from build123d import *

# Parameters (mm, degrees)
BOSS_EXTRUDE1_DEPTH = 6
SKETCH2_W           = 2.25
SKETCH2_H           = 2
CUT_EXTRUDE1_DEPTH  = 9.628586211
SKETCH3_W           = 2.25
SKETCH3_H           = 2
CUT_EXTRUDE2_DEPTH  = 9.628586211
SKETCH4_W           = 2.5
SKETCH4_H           = 50
CHAMFER1_SIZE       = 0.4905
FILLET1_R           = 0.5
FILLET2_R           = 3


with BuildPart() as part:
    # Sketch1 → Boss-Extrude1 (new body)
    with BuildSketch(Plane(origin=(0, 0, -3), x_dir=(-1, 0, 0), z_dir=(0, 0, -1))):
        Polygon((5.25, 2), (-5.25, 2), (-5.25, -1.65), (-3.6, -3.3), (3.6, -3.3), (5.25, -1.65), align=None)
    extrude(amount=-BOSS_EXTRUDE1_DEPTH)

    # Sketch2 → Cut-Extrude1 (cut, through all)
    with BuildSketch(Plane.XY.offset(3)):
        with Locations((-4.125, 1)):
            Rectangle(SKETCH2_W, SKETCH2_H)
    extrude(amount=-CUT_EXTRUDE1_DEPTH, mode=Mode.SUBTRACT)

    # Sketch3 → Cut-Extrude2 (cut, through all)
    with BuildSketch(Plane.XY.offset(3)):
        with Locations((4.125, 1)):
            Rectangle(SKETCH3_W, SKETCH3_H)
    extrude(amount=-CUT_EXTRUDE2_DEPTH, mode=Mode.SUBTRACT)

    # Sketch4 → Revolve1 (revolve)
    with BuildSketch(Plane(origin=(0, 0, 0), x_dir=(-1, 0, 0), z_dir=(0, 0, -1)), mode=Mode.PRIVATE) as revolve1_sk:
        with Locations((-1.25, 27)):
            Rectangle(SKETCH4_W, SKETCH4_H)
    revolve(revolve1_sk.sketch.rotate(Axis((0, 2, 0), (0, 1, 0)), 180), axis=Axis((0, 2, 0), (0, 1, 0)))

    # Chamfer1
    chamfer1_edges = [part.edges().sort_by_distance(p)[0] for p in [
        (2.5, 52, 0),
    ]]
    chamfer(chamfer1_edges, length=CHAMFER1_SIZE)

    # Fillet1
    fillet1_edges = [part.edges().sort_by_distance(p)[0] for p in [
        (5.25, -0.825, 3),
        (-5.25, -0.825, -3),
    ]]
    fillet(fillet1_edges, radius=FILLET1_R)

    # Fillet2
    fillet2_edges = [part.edges().sort_by_distance(p)[0] for p in [
        (-3, 1, -3),
        (3, 1, 3),
    ]]
    fillet(fillet2_edges, radius=FILLET2_R)


solid = part.part
Geometry check sheet. Reference: the model listing, model coordinates, mm. A direction names the side the tool comes from. Coordinates: 2 decimals unless noted, no trailing zeros. Order: outer loops, then holes, each group sorted by start corner. A loop starts at its lowest first (then second) coordinate and runs counter-clockwise, first axis right, second up. Notation, with made-up numbers: (-16, -10) - (43, -10) arc R10 ccw to (43, 4) - close; hole circle Ø8 at (44, -21). An arc over 180 degrees is marked (long way). One line per item, written item: value.
(1) Access from +Z, -Z, +X, -X, +Y, -Y to the whole of each face (thin tool, end or side, straight path). Record for faces 1 (the face through (2.5, 27.1, 0.1)), 2 (the face through (3, 1, -1)), 3 (the face through (2.14, 1.01, 2.1)), 4 (the face through (-3, 1, 2)).
Data:
face 1: +Y
face 2: +Z, -Z, +X, +Y
face 3: +Z, +X, +Y
face 4: +Z, -Z, -X, +Y
(2) Thickness scan on probe 1 along Y at (x, z) = (-3, -1); probe 2 along Z at (x, y) = (0, 24.5); probe 3 along Y at (x, z) = (-2.25, 2.75). Record the ranges inside material, lowest first. Write a range as from..to.
Data:
probe 1: y = -3.3..0
probe 2: z = -2.5..2.5
probe 3: y = -3.3..2
(3) Depth check by flat-ended pin: pin 1 Ø2 at (x, y) = (1, 33) entering from -Z; pin 2 Ø6 at (x, y) = (2, 38) entering from +Z; pin 3 Ø2 at (y, z) = (26, 0.5) entering from +X. Enter the tip coordinate at first touch or a pass-through.
Data:
pin 1: stops at z = -2.5
pin 2: stops at z = 2.5
pin 3: stops at x = 2.5
(4) Sectioned sample at A-A (y = 44.5). Enter the section's corners in (x, z), and give its area (3 significant figures).
Data:
outline: circle Ø5 at (0, 0)
area: 19.6 mm^2
